Here's the drawing with two shaded views (mm, measured from the low corner). I have some questions. Coordinates: 2 decimals unless noted, no trailing zeros. Order: outer loops, then holes, each group sorted by start corner. A loop starts at its lowest first (then second) coordinate and runs counter-clockwise, first axis right, second up. Notation, with made-up numbers: (9, -22.75) -> (17, -22.75) arc R24 cw to (17, 8.25) -> close; hole circle Ø7 at (-35.75, 44). An arc over 180 degrees is marked (long way). Answer in a Markdown table with one row per item. Add a question column.
1. Imagine slicing it at C-C on z = 14.5. Write out the boundary of the cut face in (x, y), plus the area to 3 significant figures.
2. If I drill on line 1 along Y through (x, z) = (21.5, 3.5); line 2 along X through (y, z) = (13, 26); line 3 along Y through (x, z) = (20, 10.5), over which ranges is the centre line in solid material (lowest first)? Write a range as [from, to].
3. We'd pull the mould along Y, two halves only. Please class the marked faces 1, 2, 3 and 4: pulls with the +Y half, pulls with the -Y half, needs draft (parallel to the pull), parting line crosses it, or undercut.
4. Imagine slicing it at A-A on x = 20. Write out the boundary of the cut face in (y, z), plus the area to 3 significant figures.
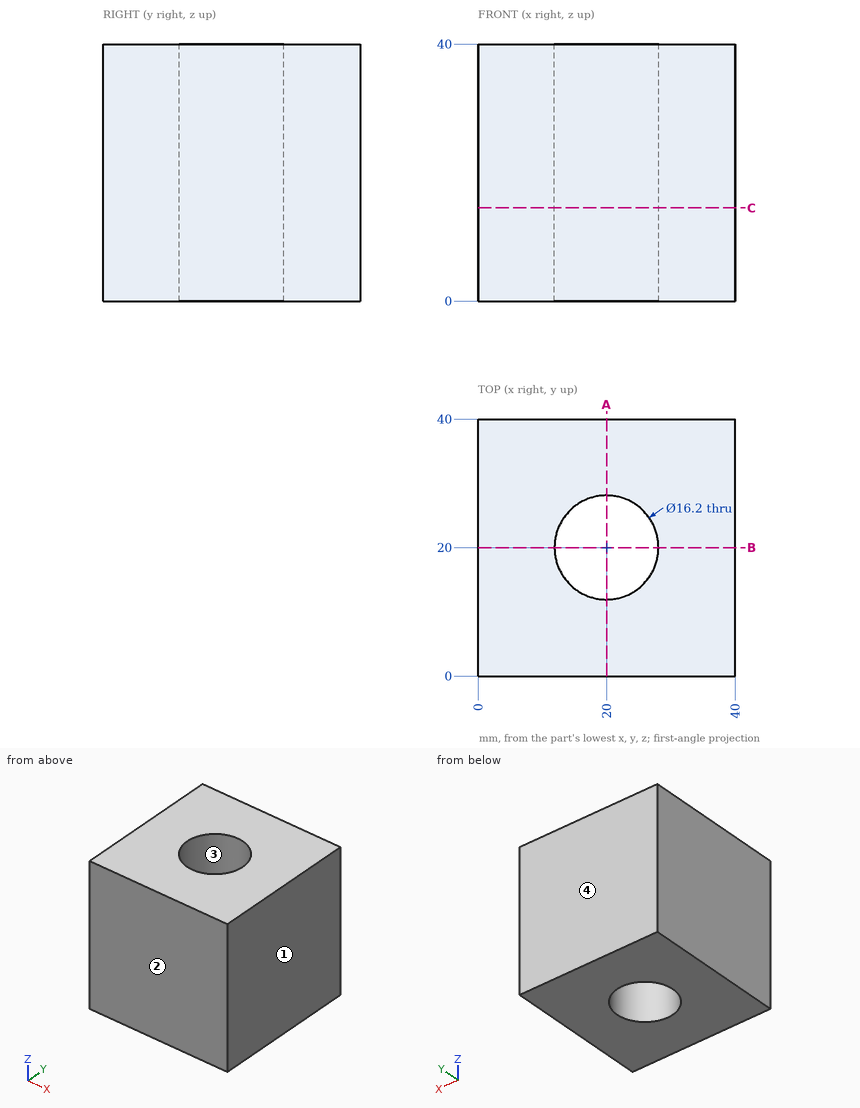
Answers follow:
| question | item | result |
|---|---|---|
| 1 | outline | (0, 0) -> (40, 0) -> (40, 40) -> (0, 40) -> close; hole circle Ø16.2 at (20, 20) |
| 1 | area | 1,390 mm² |
| 2 | line 1 | y = [0, 12.04], [27.96, 40] |
| 2 | line 2 | x = [0, 15.92], [24.08, 40] |
| 2 | line 3 | y = [0, 11.9], [28.1, 40] |
| 3 | face 1 | needs draft |
| 3 | face 2 | pulls with the -Y half |
| 3 | face 3 | undercut |
| 3 | face 4 | pulls with the +Y half |
| 4 | outline | (0, 0) -> (11.9, 0) -> (11.9, 40) -> (0, 40) -> close; (28.1, 0) -> (40, 0) -> (40, 40) -> (28.1, 40) -> close |
| 4 | area | 952 mm² |
